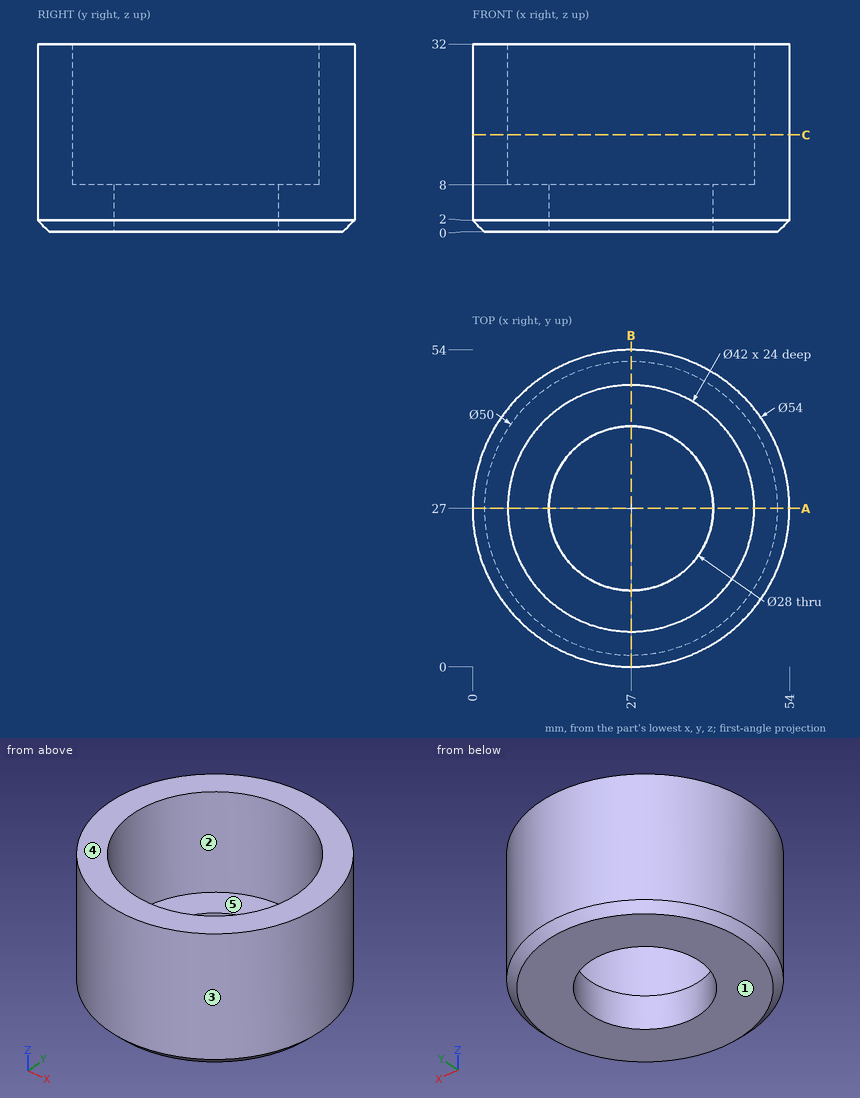
Geometry: see drawing. Coordinates: mm, zero at the bounding-box minimum. A direction names the side the tool comes from. Give positions to 0.01 mm unless a question says otherwise; leave off trailing zeros. Loops run counter-clockwise (first coordinate to the right, second up) from the corner with the lowest first, then second, coordinate; pieces in that order, holes last. Notation, with made-up numbers: M 20,17.25 L 57,17.25 A22 cw 57,47.25 Z; hole C -40,-20.75 d11. An arc over 180 degrees is marked long. Answer as CSV lines item,"result". Start each with the question number.
1. Section C-C on z = 16.5. Return loops of the section in (x, y).
2. Section A-A on y = 27. Return loops of the section in (x, z).
3. Line query: L1, parallel to Y at x = 27, z = 4; L2, parallel to Z at x = 25.5, y = 7; L3, parallel to Y at x = 24, z = 26.5. Output: solid intervals per line, ascending.
4. Pull-direction query (X, two-part tool) for the marked faces 3, 4 and 5; classes: released by +X, released by -X, zero draft, split by the parting line, or undercut.
5. Pin query (flat end, axial travel): P1, Ø1, axis at x = 18, z = 20.5, coming from the -Y side; P2, Ø2, axis at x = 23.5, y = 44, coming from the +Z side; P3, Ø4, axis at x = 15, z = 10, coming from the +Y side. Return the tip coordinate at first contact, or that it passes through.
6. Reachability of the marked faces 1 and 2 from +Z, -Z, +X, -X, +Y, -Y: full face, straight path, thin tool, end or side. Return the list, or none.
Computed values:
1,outline,"C 27,27 d54; hole C 27,27 d42"
2,outline,"M 0,2 L 2,0 L 13,0 L 13,8 L 6,8 L 6,32 L 0,32 Z; M 41,0 L 52,0 L 54,2 L 54,32 L 48,32 L 48,8 L 41,8 Z"
3,L1,"y = 0 to 13, 41 to 54"
3,L2,"z = 0 to 8"
3,L3,"y = 0.17 to 6.22, 47.78 to 53.83"
4,face 3,"split by the parting line"
4,face 4,"zero draft"
4,face 5,"undercut"
5,P1,"stops at y = 1.37"
5,P2,"stops at z = 8"
5,P3,"stops at y = 52.08"
6,face 1,"-Z, +X, -X, +Y, -Y"
6,face 2,"+Z"
